from build123d import *

# Parameters (mm, degrees)
BOSS_EXTRUDE1_DEPTH = 4
SKETCH2_R           = 2
SKETCH2_R_2         = 1.5
BOSS_EXTRUDE2_DEPTH = 3


with BuildPart() as part:
    # Sketch1 → Boss-Extrude1 (new, symmetric)
    with BuildSketch(Plane(origin=(0, 0, 0), x_dir=(1, 0, 0), z_dir=(0, 1, 0))):
        with BuildLine():
            Line((7, 0), (-7, 0))
            Line((-7, 0), (-6, -5))
            ThreePointArc((-6, -5), (0, -4.547439867), (6, -5))
            Line((6, -5), (7, 0))
        make_face()
    extrude(amount=BOSS_EXTRUDE1_DEPTH, both=True)

    # Sketch2 → Boss-Extrude2 (add)
    with BuildSketch(Plane.XY):
        Circle(SKETCH2_R)
        Circle(SKETCH2_R_2, mode=Mode.SUBTRACT)
    extrude(amount=-BOSS_EXTRUDE2_DEPTH)


solid = part.part
Work out the finished part from the listing and answer in its coordinate system (mm). A direction names the side the tool comes from. Round coordinates to 2 decimals unless told otherwise and drop trailing zeros. Order: outer loops, then holes, each group sorted by start corner. A loop starts at its lowest first (then second) coordinate and runs counter-clockwise, first axis right, second up. Notation, with made-up numbers: M 5.5,48.5 L 63.5,48.5 A17 ccw 63.5,73.5 Z; hole C 6.5,-34.75 d8. An arc over 180 degrees is marked long. Put each result on its own line as item: value. Start each with the question number.
Q1. Straight lines are drawn through the part: L1, parallel to Y at x = 0, z = -1.4; L2, parallel to Z at x = 0.5, y = 2.75. For each, find the intervals that lie inside material, in ascending order. Write a range as [from, to].
Q2. Flat-ended cylindrical pins translate along their axes: pin 1 (2.5 mm diameter, centred on x = 0, y = 0, fed in from +Z); pin 2 (1.5 mm diameter, centred on x = -2, y = -2, fed in from -Z). Find the tip coordinate at first contact, or state that the pin passes through.
Q3. A tool of negligible diameter and unlimited length cuts with its end or side. For faces 5 (the flat face through (-6.5, 0.1, 2.5)), 6 (the cylindrical face through (0, -2, -1)), from which of +Z, -Z, +X, -X, +Y, -Y can it reach the whole face along a straight path? Write none if from no direction.
Q4. Section B-B, the plane y = 0 is taken. Write down the section's boundary in (x, z), and give its area (3 significant figures).
Q5. Section D-D, the plane x = -1.75 is taken. Write down the section's boundary in (y, z).
Q6. For a pull along X with two mould halves and no side action, classify faces 1 (the cylindrical face through (-1.5, 0.07, -1.48)), 2 (the flat face through (0, 0, 0)), 3 (the flat face through (6.5, 0.1, 2.5)), 4 (the flat face through (0, -4, 2)) as pulls with the +X half, pulls with the -X half, needs draft (parallel to the pull), parting line crosses it, or undercut.
Q7. Section C-C, the plane z = 2 is taken. Write down the section's boundary in (x, y).
Q8. Section A-A, the plane x = 0 is taken. Write down the section's boundary in (y, z), and give its area (3 significant figures).
Findings below:
1. L1: y = [-2, -1.5], [1.5, 2]
1. L2: z = [0, 4.55]
2. pin 1: stops at z = 4.57
2. pin 2: stops at z = 0
3. face 5: +Z, -X, +Y, -Y
3. face 6: -Z
4. outline: M -7,0 L -2,0 L -2,-3 L -1.5,-3 L -1.5,0 L 1.5,0 L 1.5,-3 L 2,-3 L 2,0 L 7,0 L 6,5 A40 cw -6,5 Z
4. area: 64.4 mm^2
5. outline: M -4,0 L -0.97,0 L -0.97,-3 L 0.97,-3 L 0.97,0 L 4,0 L 4,4.59 L -4,4.59 Z
6. face 1: undercut
6. face 2: undercut
6. face 3: pulls with the +X half
6. face 4: needs draft
7. outline: M -6.6,-4 L 6.6,-4 L 6.6,4 L -6.6,4 Z
8. outline: M -4,0 L -2,0 L -2,-3 L -1.5,-3 L -1.5,0 L 1.5,0 L 1.5,-3 L 2,-3 L 2,0 L 4,0 L 4,4.55 L -4,4.55 Z
8. area: 39.4 mm^2
